CAD build for the part. Positions are in the model's coordinates, mm. Face numbers are marked on the shaded views. A direction names the side the tool comes from. Give positions to 0.01 mm unless a question says otherwise; leave off trailing zeros. Write each loop counter-clockwise with the first axis right and the second up, starting at its lowest first coordinate (ties: lowest second). Pieces come first, ordered by that corner, then holes. Notation, with made-up numbers: (-13, 11.25) - (23, 11.25) arc R16 cw to (23, 35.25) - close; hole circle Ø10 at (73, 23.25). An arc over 180 degrees is marked (long way). Answer as a JSON object with one key per item and string values.
from build123d import *

# Parameters (mm, degrees)
BASE_PLATE_SKETCH_W              = 62
BASE_PLATE_SKETCH_H              = 50
BASE_PLATE_62X50X12_DEPTH        = 12
COLUMN_SKETCH_W                  = 18
COLUMN_SKETCH_H                  = 50
COLUMN_9X9_DEPTH                 = 70
UPPER_HUB_DEPTH                  = 3
UPPER_HUB_DEPTH_BACK             = 43
UPPER_HUB_SKETCH_R               = 25
UPPER_HUB_SKETCH_R_2             = 12.5
LOWER_EAR_A_BLOCK_SKETCH_W       = 50
LOWER_EAR_A_BLOCK_SKETCH_H       = 28
LOWER_EAR_A_BLOCK_DEPTH          = 15
LOWER_EAR_A_ROUND_END_DEPTH      = 3
LOWER_EAR_A_ROUND_END_DEPTH_BACK = 15
LOWER_EAR_A_ROUND_END_SKETCH_R   = 28
LOWER_EAR_A_ROUND_END_SKETCH_R_2 = 16
LOWER_EAR_A_PIN_HOLE_SKETCH_R    = 16
LOWER_EAR_A_PIN_HOLE_DEPTH       = 15
LOWER_EAR_B_BLOCK_SKETCH_W       = 50
LOWER_EAR_B_BLOCK_SKETCH_H       = 28
LOWER_EAR_B_BLOCK_DEPTH          = 15
LOWER_EAR_B_ROUND_END_DEPTH      = 3
LOWER_EAR_B_ROUND_END_DEPTH_BACK = 15
LOWER_EAR_B_ROUND_END_SKETCH_R   = 28
LOWER_EAR_B_ROUND_END_SKETCH_R_2 = 16
LOWER_START                      = -15
LOWER_EAR_B_PIN_HOLE_SKETCH_R    = 16
LOWER_EAR_B_PIN_HOLE_DEPTH       = 15
UPPER_BRACKET_BLOCK_DEPTH        = 25
UPPER_BRACKET_BLOCK_DEPTH_BACK   = 25
UPPER_BRACKET_BLOCK_SKETCH_W     = 18
UPPER_BRACKET_BLOCK_SKETCH_H     = 36
UPPER_CLEVIS_ARM_SKETCH_W        = 42
UPPER_CLEVIS_ARM_SKETCH_H        = 36
UPPER_CLEVIS_ARM_DEPTH           = 30
CLEVIS_SLOT_SKETCH_W             = 18
CLEVIS_SLOT_SKETCH_H             = 36
CLEVIS_SLOT_12X12_DEPTH          = 18
UPPER_EAR_A_ROUND_END_DEPTH      = 3
UPPER_EAR_A_ROUND_END_DEPTH_BACK = 12
UPPER_EAR_A_ROUND_END_SKETCH_R   = 18.096202238
UPPER_EAR_A_ROUND_END_SKETCH_R_2 = 7.5
UPPER_EAR_A_PIN_HOLE_SKETCH_R    = 7.5
UPPER_EAR_A_PIN_HOLE_DEPTH       = 12
UPPER_EAR_B_ROUND_END_DEPTH      = 3
UPPER_EAR_B_ROUND_END_DEPTH_BACK = 12
UPPER_EAR_B_ROUND_END_SKETCH_R   = 18
UPPER_EAR_B_ROUND_END_SKETCH_R_2 = 7.5
UPPER_START                      = -12
UPPER_EAR_B_PIN_HOLE_SKETCH_R    = 7.5
UPPER_EAR_B_PIN_HOLE_DEPTH       = 12
HUB_BORE_SKETCH_R                = 12.5
HUB_BORE_THROUGH_DEPTH           = 66


with BuildPart() as part:
    # Base Plate Sketch → Base Plate 62x50x12 (new body)
    with BuildSketch(Plane(origin=(0, 0, 0), x_dir=(1, 0, 0), z_dir=(0, 1, 0))):
        Rectangle(BASE_PLATE_SKETCH_W, BASE_PLATE_SKETCH_H)
    extrude(amount=BASE_PLATE_62X50X12_DEPTH)

    # Column Sketch → Column 9x9 (add)
    with BuildSketch(Plane(origin=(0, 12, 0), x_dir=(1, 0, 0), z_dir=(0, 1, 0))):
        Rectangle(COLUMN_SKETCH_W, COLUMN_SKETCH_H)
    extrude(amount=COLUMN_9X9_DEPTH)

    # Upper Hub Sketch → Upper Hub (add, two sides: drawn at the far end of the back side and taken through both)
    with BuildSketch(Plane(origin=(9, 0, 0), x_dir=(0, 0, -1), z_dir=(1, 0, 0)).offset(-UPPER_HUB_DEPTH_BACK)):
        with Locations((0, 82)):
            Circle(UPPER_HUB_SKETCH_R)
        with Locations((0, 82)):
            Circle(UPPER_HUB_SKETCH_R_2, mode=Mode.SUBTRACT)
    extrude(amount=UPPER_HUB_DEPTH + UPPER_HUB_DEPTH_BACK)

    # Lower Ear A Block Sketch → Lower Ear A Block (add)
    with BuildSketch(Plane(origin=(31, 0, 0), x_dir=(0, 0, -1), z_dir=(1, 0, 0))):
        with Locations((0, -14)):
            Rectangle(LOWER_EAR_A_BLOCK_SKETCH_W, LOWER_EAR_A_BLOCK_SKETCH_H)
    extrude(amount=-LOWER_EAR_A_BLOCK_DEPTH)

    # Lower Ear A Round End Sketch → Lower Ear A Round End (add, two sides: drawn at the far end of the back side and taken through both)
    with BuildSketch(Plane(origin=(31, 0, 0), x_dir=(0, 0, -1), z_dir=(1, 0, 0)).offset(-LOWER_EAR_A_ROUND_END_DEPTH_BACK)):
        with Locations(Location((0, -28, 0), (0, 0, 153.234499423))):
            Circle(LOWER_EAR_A_ROUND_END_SKETCH_R)
        with Locations((0, -28)):
            Circle(LOWER_EAR_A_ROUND_END_SKETCH_R_2, mode=Mode.SUBTRACT)
    extrude(amount=LOWER_EAR_A_ROUND_END_DEPTH + LOWER_EAR_A_ROUND_END_DEPTH_BACK)

    # Lower Ear A Pin Hole Sketch → Lower Ear A Pin Hole (cut)
    with BuildSketch(Plane(origin=(31, 0, 0), x_dir=(0, 0, -1), z_dir=(1, 0, 0))):
        with Locations((0, -28)):
            Circle(LOWER_EAR_A_PIN_HOLE_SKETCH_R)
    extrude(amount=-LOWER_EAR_A_PIN_HOLE_DEPTH, mode=Mode.SUBTRACT)

    # Lower Ear B Block Sketch → Lower Ear B Block (add)
    with BuildSketch(Plane.ZY.offset(31)):
        with Locations((0, -14)):
            Rectangle(LOWER_EAR_B_BLOCK_SKETCH_W, LOWER_EAR_B_BLOCK_SKETCH_H)
    extrude(amount=-LOWER_EAR_B_BLOCK_DEPTH)

    # Lower Ear B Round End Sketch → Lower Ear B Round End (add, two sides: drawn at the far end of the back side and taken through both)
    with BuildSketch(Plane.ZY.offset(31).offset(-LOWER_EAR_B_ROUND_END_DEPTH_BACK)):
        with Locations(Location((0, -28, 0), (0, 0, 26.765500577))):
            Circle(LOWER_EAR_B_ROUND_END_SKETCH_R)
        with Locations(Location((0, -28, 0), (0, 0, 180))):
            Circle(LOWER_EAR_B_ROUND_END_SKETCH_R_2, mode=Mode.SUBTRACT)
    extrude(amount=LOWER_EAR_B_ROUND_END_DEPTH + LOWER_EAR_B_ROUND_END_DEPTH_BACK)

    # Lower Ear B Pin Hole Sketch → Lower Ear B Pin Hole (cut)
    with BuildSketch(Plane.ZY.offset(31).offset(LOWER_START)):
        with Locations(Location((0, -28, 0), (0, 0, 180))):
            Circle(LOWER_EAR_B_PIN_HOLE_SKETCH_R)
    extrude(amount=LOWER_EAR_B_PIN_HOLE_DEPTH, mode=Mode.SUBTRACT)

    # Upper Bracket Block Sketch → Upper Bracket Block (add, two sides: drawn at the far end of the back side and taken through both)
    with BuildSketch(Plane.XY.offset(25).offset(-UPPER_BRACKET_BLOCK_DEPTH_BACK)):
        with Locations((-11, 89)):
            Rectangle(UPPER_BRACKET_BLOCK_SKETCH_W, UPPER_BRACKET_BLOCK_SKETCH_H)
    extrude(amount=UPPER_BRACKET_BLOCK_DEPTH + UPPER_BRACKET_BLOCK_DEPTH_BACK)

    # Upper Clevis Arm Sketch → Upper Clevis Arm (add)
    with BuildSketch(Plane.XY.offset(50)):
        with Locations((-11, 89)):
            Rectangle(UPPER_CLEVIS_ARM_SKETCH_W, UPPER_CLEVIS_ARM_SKETCH_H)
    extrude(amount=UPPER_CLEVIS_ARM_DEPTH)

    # Clevis Slot Sketch → Clevis Slot 12x12 (cut)
    with BuildSketch(Plane.XY.offset(80)):
        with Locations((-11, 89)):
            Rectangle(CLEVIS_SLOT_SKETCH_W, CLEVIS_SLOT_SKETCH_H)
    extrude(amount=-CLEVIS_SLOT_12X12_DEPTH, mode=Mode.SUBTRACT)

    # Upper Ear A Round End Sketch → Upper Ear A Round End (add, two sides: drawn at the far end of the back side and taken through both)
    with BuildSketch(Plane(origin=(10, 0, 0), x_dir=(0, 0, -1), z_dir=(1, 0, 0)).offset(-UPPER_EAR_A_ROUND_END_DEPTH_BACK)):
        with Locations(Location((-80, 89, 0), (0, 0, 275.910566162))):
            Circle(UPPER_EAR_A_ROUND_END_SKETCH_R)
        with Locations(Location((-80, 89, 0), (0, 0, 90))):
            Circle(UPPER_EAR_A_ROUND_END_SKETCH_R_2, mode=Mode.SUBTRACT)
    extrude(amount=UPPER_EAR_A_ROUND_END_DEPTH + UPPER_EAR_A_ROUND_END_DEPTH_BACK)

    # Upper Ear A Pin Hole Sketch → Upper Ear A Pin Hole (cut)
    with BuildSketch(Plane(origin=(10, 0, 0), x_dir=(0, 0, -1), z_dir=(1, 0, 0))):
        with Locations(Location((-80, 89, 0), (0, 0, 90))):
            Circle(UPPER_EAR_A_PIN_HOLE_SKETCH_R)
    extrude(amount=-UPPER_EAR_A_PIN_HOLE_DEPTH, mode=Mode.SUBTRACT)

    # Upper Ear B Round End Sketch → Upper Ear B Round End (add, two sides: drawn at the far end of the back side and taken through both)
    with BuildSketch(Plane.ZY.offset(32).offset(-UPPER_EAR_B_ROUND_END_DEPTH_BACK)):
        with Locations(Location((80, 89, 0), (0, 0, 270))):
            Circle(UPPER_EAR_B_ROUND_END_SKETCH_R)
        with Locations(Location((80, 89, 0), (0, 0, 90))):
            Circle(UPPER_EAR_B_ROUND_END_SKETCH_R_2, mode=Mode.SUBTRACT)
    extrude(amount=UPPER_EAR_B_ROUND_END_DEPTH + UPPER_EAR_B_ROUND_END_DEPTH_BACK)

    # Upper Ear B Pin Hole Sketch → Upper Ear B Pin Hole (cut)
    with BuildSketch(Plane.ZY.offset(32).offset(UPPER_START)):
        with Locations(Location((80, 89, 0), (0, 0, 90))):
            Circle(UPPER_EAR_B_PIN_HOLE_SKETCH_R)
    extrude(amount=UPPER_EAR_B_PIN_HOLE_DEPTH, mode=Mode.SUBTRACT)

    # Hub Bore Sketch → Hub Bore Through (cut)
    with BuildSketch(Plane.ZY.offset(34)):
        with Locations(Location((0, 82, 0), (0, 0, 180))):
            Circle(HUB_BORE_SKETCH_R)
    extrude(amount=-HUB_BORE_THROUGH_DEPTH, mode=Mode.SUBTRACT)


solid = part.part
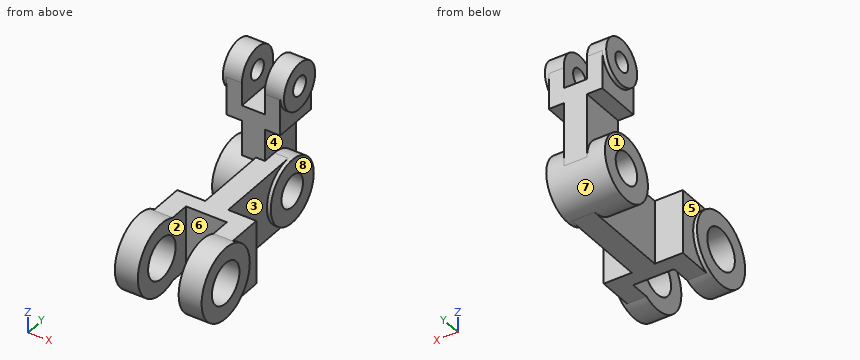
(1) Saw through at D-D, the plane z = -10.5. State how many separate pieces and enclosed holes the cut face has, and give its area (3 significant figures).
Answer key:
{"separate pieces": "4", "enclosed holes": "0", "area": "4,120 mm²"}
(2) 3-axis set-ups, long thin cutter, end or side, ignore diameter. For the marked faces 4, 5, 6, 7 and 8: which of +Z, -Z, +X, -X, +Y, -Y reach the whole face in a straight line?
Answer key:
{"face 4": "+X, +Y", "face 5": "-X", "face 6": "+Z, -Z, -Y", "face 7": "none", "face 8": "-Z, +X, +Y"}
(3) Saw through at A-A, the plane x = -25. Give the cut face in (y, z), and give its area (3 significant figures).
Answer key:
{"outline": "(-15.39, -25) - (12, -25) - (12, 25) - (-15.39, 25) arc R28 ccw (long way) to start; circle Ø50 at (82, 0); (71, 50) - (107, 50) - (107, 80) arc R18 ccw to (71, 80) - close; hole circle Ø32 at (-28, 0); hole circle Ø25 at (82, 0); hole circle Ø15 at (89, 80)", "area": "5,360 mm²"}
(4) Probe L1, parallel to Y at x = -22, z = 0; L2, parallel to Z at x = 9, y = 89; L3, parallel to X at y = -3, z = -9. List the from-to ranges inside material, lowest first. Write a range as [from, to].
Answer key:
{"L1": "y = [-56, -44], [-12, 12], [57, 69.5], [94.5, 107]", "L2": "z = [-24, -10.36], [10.36, 24], [50, 72.5], [87.5, 98.1]", "L3": "x = [-34, -16], [16, 34]"}
(5) Saw through at C-C, the plane y = -9. Give the cut face in (x, z).
Answer key:
{"outline": "(-34, -20.57) - (-31, -20.57) - (-31, -25) - (-16, -25) - (-16, 25) - (-31, 25) - (-31, 20.57) - (-34, 20.57) - close; (16, -25) - (31, -25) - (31, -20.57) - (34, -20.57) - (34, 20.57) - (31, 20.57) - (31, 25) - (16, 25) - close"}
(6) Saw through at B-B, the plane x = 4.5. Give the cut face in (y, z).
Answer key:
{"outline": "(0, -25) - (82, -25) arc R25 ccw to (82, 25) - (0, 25) - close; (71, 50) - (107, 50) - (107, 78.14) arc R18.1 ccw (long way) to (71, 78.14) - close; hole circle Ø25 at (82, 0); hole circle Ø15 at (89, 80)"}
(7) Pull direction X, two halves, no side cores. Call the marked faces 1, 2 and 3: pulls with the +X half, pulls with the -X half, needs draft (parallel to the pull), parting line crosses it, or undercut.
Answer key:
{"face 1": "pulls with the -X half", "face 2": "undercut", "face 3": "pulls with the +X half"}
(8) Flat gauge pins, fed straight in: P1, Ø3, axis at x = 4, z = 58, coming from the -Y side; P2, Ø3, axis at y = 28.5, z = 8, coming from the -X side; P3, Ø19.5, axis at y = 89, z = 80, coming from the +X side. Where does each tip first touch, or does it go through?
Answer key:
{"P1": "stops at y = 71", "P2": "stops at x = -9", "P3": "stops at x = 13"}
